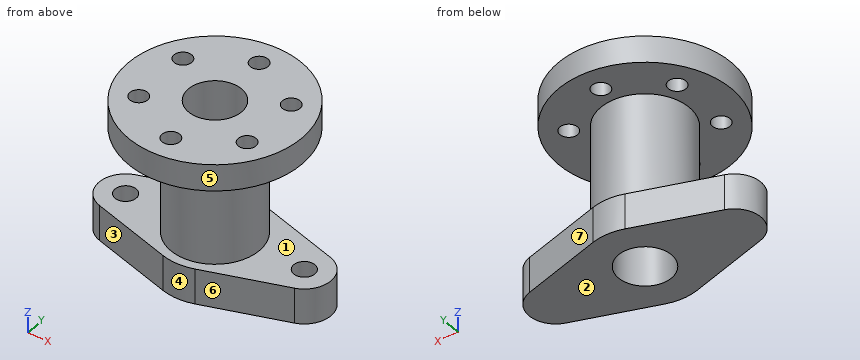
```python
from build123d import *

# Parameters (mm, degrees)
MOUNTING_PLATE_DEPTH              = 20
HUB_SKETCH_R                      = 25
HUB_50_DEPTH                      = 60
FLANGE_SKETCH_R                   = 49
FLANGE_98_DEPTH                   = 15
FLANGE_BOLT_HOLE_SKETCH_R         = 5
FLANGE_BOLT_HOLE_10_DEPTH         = 15
BORE_SKETCH_R                     = 15
BORE_CUT_DEPTH                    = 158.006369298
FLANGE_BOLT_HOLE_PATTERN_6X_COUNT = 6
PLATE_HOLES_SKETCH_R              = 6
PLATE_HOLES_2X_12_DEPTH           = 15


with BuildPart() as part:
    # Mounting Plate Sketch → Mounting Plate (new body)
    with BuildSketch(Plane.XY):
        with BuildLine():
            Line((-4.5, 14.309088021), (41, 28.618176043))
            ThreePointArc((41, 28.618176043), (50, 30), (59, 28.618176043))
            Line((59, 28.618176043), (104.5, 14.309088021))
            ThreePointArc((104.5, 14.309088021), (115, 0), (104.5, -14.309088021))
            Line((104.5, -14.309088021), (59, -28.618176043))
            ThreePointArc((59, -28.618176043), (50, -30), (41, -28.618176043))
            Line((41, -28.618176043), (-4.5, -14.309088021))
            ThreePointArc((-4.5, -14.309088021), (-15, 0), (-4.5, 14.309088021))
        make_face()
    extrude(amount=MOUNTING_PLATE_DEPTH)

    # Hub Sketch → Hub Ø50 (add)
    with BuildSketch(Plane.XY.offset(20)):
        with Locations((50, 0)):
            Circle(HUB_SKETCH_R)
    extrude(amount=HUB_50_DEPTH)

    # Flange Sketch → Flange Ø98 (add)
    with BuildSketch(Plane.XY.offset(80)):
        with Locations((50, 0)):
            Circle(FLANGE_SKETCH_R)
    extrude(amount=FLANGE_98_DEPTH)

    # Flange Bolt Hole Sketch → Flange Bolt Hole Ø10 (cut)
    with BuildSketch(Plane.XY.offset(95)):
        with Locations((50, 35)):
            Circle(FLANGE_BOLT_HOLE_SKETCH_R)
    flange_bolt_hole_10 = extrude(amount=-FLANGE_BOLT_HOLE_10_DEPTH, mode=Mode.SUBTRACT)

    # Bore Sketch → Bore Cut (cut, through all)
    with BuildSketch(Plane.XY.offset(95)):
        with Locations((50, 0)):
            Circle(BORE_SKETCH_R)
    extrude(amount=-BORE_CUT_DEPTH, mode=Mode.SUBTRACT)

    # Flange Bolt Hole Pattern 6x: Flange Bolt Hole Ø10 ×6 about axis
    flange_bolt_hole_pattern_6x_axis = Axis((50, 0, 0), (0, 0, 1))
    for i in range(1, FLANGE_BOLT_HOLE_PATTERN_6X_COUNT):
        add(flange_bolt_hole_10.rotate(flange_bolt_hole_pattern_6x_axis, i * 360 / FLANGE_BOLT_HOLE_PATTERN_6X_COUNT), mode=Mode.SUBTRACT)

    # Plate Holes Sketch → Plate Holes 2xØ12 (cut)
    with BuildSketch(Plane.XY.offset(20)):
        Circle(PLATE_HOLES_SKETCH_R)
        with Locations((100, 0)):
            Circle(PLATE_HOLES_SKETCH_R)
    extrude(amount=-PLATE_HOLES_2X_12_DEPTH, mode=Mode.SUBTRACT)


solid = part.part
```
Geometry check sheet. Reference: the model listing, model coordinates, mm. Face numbers are marked on the shaded views. A direction names the side the tool comes from. Coordinates: 2 decimals unless noted, no trailing zeros. Order: outer loops, then holes, each group sorted by start corner. A loop starts at its lowest first (then second) coordinate and runs counter-clockwise, first axis right, second up. Notation, with made-up numbers: (59, 38) - (94, 38) arc R34 ccw to (94, 69) - close; hole circle Ø5 at (59.5, -36). An arc over 180 degrees is marked (long way). Answer in a Markdown table with one row per item. Add a question column.
1. Section check B-B (y = 8). Enter the section's corners in (x, z).
2. Section check D-D (y = -17.5). Enter the section's corners in (x, z).
3. Material ranges on L1, parallel to Z at x = 48.5, y = -27; L2, parallel to X at y = -2.5, z = 25; L3, parallel to Z at x = 25, y = -30, recorded low to high. Write a range as [from, to].
4. Section check C-C (z = 56). Enter the section's corners in (x, y).
5. Access from +Z, -Z, +X, -X, +Y, -Y to the whole of each face (thin tool, end or side, straight path). Record for the marked faces 4, 5, 6 and 7.
6. Section check A-A (x = 50). Enter the section's corners in (y, z), plus the area to 3 significant figures.
7. Draft check along Z on the marked faces 1, 2 and 3. Enter one of: +Z half, -Z half, draft (parallel to the pull), parting line (faces both ways), or undercut.
8. Gauge pin test, flat ends, axial feed: pin 1 Ø5 at (x, z) = (67, 70) entering from -Y; pin 2 Ø2 at (x, z) = (68.5, 54) entering from +Y; pin 3 Ø6 at (y, z) = (34, 15) entering from +X; pin 4 Ø3.5 at (x, y) = (-1.5, -1.5) entering from +Z. Record the tip position at first contact, or that the pin passes through.
Data:
| question | item | result |
|---|---|---|
| 1 | outline | (-12.69, 0) - (37.31, 0) - (37.31, 95) - (1.66, 95) - (1.66, 80) - (26.31, 80) - (26.31, 20) - (-12.69, 20) - close; (62.69, 0) - (112.69, 0) - (112.69, 20) - (73.69, 20) - (73.69, 80) - (98.34, 80) - (98.34, 95) - (62.69, 95) - close |
| 2 | outline | (4.23, 80) - (14.69, 80) - (14.69, 95) - (4.23, 95) - close; (5.65, 0) - (94.35, 0) - (94.35, 20) - (67.85, 20) - (67.85, 80) - (75.31, 80) - (75.31, 95) - (24.69, 95) - (24.69, 80) - (32.15, 80) - (32.15, 20) - (5.65, 20) - close; (85.31, 80) - (95.77, 80) - (95.77, 95) - (85.31, 95) - close |
| 3 | L1 | z = [0, 20], [80, 95] |
| 3 | L2 | x = [25.13, 35.21], [64.79, 74.87] |
| 3 | L3 | z = [80, 95] |
| 4 | outline | circle Ø50 at (50, 0); hole circle Ø30 at (50, 0) |
| 5 | face 4 | -Z, -Y |
| 5 | face 5 | +Z |
| 5 | face 6 | -Z, +X, -Y |
| 5 | face 7 | -Z, +X, +Y |
| 6 | outline | (-49, 80) - (-40, 80) - (-40, 95) - (-49, 95) - close; (-30, 0) - (-15, 0) - (-15, 95) - (-30, 95) - (-30, 80) - (-25, 80) - (-25, 20) - (-30, 20) - close; (15, 0) - (30, 0) - (30, 20) - (25, 20) - (25, 80) - (30, 80) - (30, 95) - (15, 95) - close; (40, 80) - (49, 80) - (49, 95) - (40, 95) - close |
| 6 | area | 2,520 mm² |
| 7 | face 1 | undercut |
| 7 | face 2 | -Z half |
| 7 | face 3 | draft |
| 8 | pin 1 | stops at y = -20.37 |
| 8 | pin 2 | stops at y = 17.85 |
| 8 | pin 3 | passes through |
| 8 | pin 4 | stops at z = 5 |
